```python
from build123d import *

# Parameters (mm, degrees)
SKETCH16_R             = 3.4
SKETCH16_R_2           = 3
MEMBER_1_DEPTH         = 340
HOLE_WIZARD_M8_3_D     = 6.9
HOLE_WIZARD_M8_3_DEPTH = 19.75
HOLE_WIZARD_M8_3_TIP   = 2.072969136


with BuildPart() as part:
    # Sketch16 → Member 1 (new body)
    with BuildSketch(Plane(origin=(0, 0, 0), x_dir=(-1, 0, 0), z_dir=(0, 1, 0))):
        with BuildLine():
            Line((-5.1, 20), (-5.1, 19.5))
            Line((-5.1, 19.5), (-4.1, 19.5))
            Line((-4.1, 19.5), (-4.1, 17))
            Line((-4.1, 17), (-6.1, 17))
            Line((-6.1, 17), (-6.1, 18))
            Line((-6.1, 18), (-10.3, 18))
            Line((-10.3, 18), (-10.3, 12))
            Line((-10.3, 12), (-6, 7.7))
            Line((-6, 7.7), (6, 7.7))
            Line((6, 7.7), (10.3, 12))
            Line((10.3, 12), (10.3, 18))
            Line((10.3, 18), (6.1, 18))
            Line((6.1, 18), (6.1, 17))
            Line((6.1, 17), (4.1, 17))
            Line((4.1, 17), (4.1, 19.5))
            Line((4.1, 19.5), (5.1, 19.5))
            Line((5.1, 19.5), (5.1, 20))
            Line((5.1, 20), (15.5, 20))
            ThreePointArc((15.5, 20), (18.681980515, 18.681980515), (20, 15.5))
            Line((20, 15.5), (20, 5.1))
            Line((20, 5.1), (19.5, 5.1))
            Line((19.5, 5.1), (19.5, 4.1))
            Line((19.5, 4.1), (17, 4.1))
            Line((17, 4.1), (17, 6.1))
            Line((17, 6.1), (18, 6.1))
            Line((18, 6.1), (18, 10.3))
            Line((18, 10.3), (12, 10.3))
            Line((12, 10.3), (7.7, 6))
            Line((7.7, 6), (7.7, -6))
            Line((7.7, -6), (12, -10.3))
            Line((12, -10.3), (18, -10.3))
            Line((18, -10.3), (18, -6.1))
            Line((18, -6.1), (17, -6.1))
            Line((17, -6.1), (17, -4.1))
            Line((17, -4.1), (19.5, -4.1))
            Line((19.5, -4.1), (19.5, -5.1))
            Line((19.5, -5.1), (20, -5.1))
            Line((20, -5.1), (20, -15.5))
            ThreePointArc((20, -15.5), (18.681980515, -18.681980515), (15.5, -20))
            Line((15.5, -20), (5.1, -20))
            Line((5.1, -20), (5.1, -19.5))
            Line((5.1, -19.5), (4.1, -19.5))
            Line((4.1, -19.5), (4.1, -17))
            Line((4.1, -17), (6.1, -17))
            Line((6.1, -17), (6.1, -18))
            Line((6.1, -18), (10.3, -18))
            Line((10.3, -18), (10.3, -12))
            Line((10.3, -12), (6, -7.7))
            Line((6, -7.7), (-6, -7.7))
            Line((-6, -7.7), (-10.3, -12))
            Line((-10.3, -12), (-10.3, -18))
            Line((-10.3, -18), (-6.1, -18))
            Line((-6.1, -18), (-6.1, -17))
            Line((-6.1, -17), (-4.1, -17))
            Line((-4.1, -17), (-4.1, -19.5))
            Line((-4.1, -19.5), (-5.1, -19.5))
            Line((-5.1, -19.5), (-5.1, -20))
            Line((-5.1, -20), (-15.5, -20))
            ThreePointArc((-15.5, -20), (-18.681980515, -18.681980515), (-20, -15.5))
            Line((-20, -15.5), (-20, -5.1))
            Line((-20, -5.1), (-19.5, -5.1))
            Line((-19.5, -5.1), (-19.5, -4.1))
            Line((-19.5, -4.1), (-17, -4.1))
            Line((-17, -4.1), (-17, -6.1))
            Line((-17, -6.1), (-18, -6.1))
            Line((-18, -6.1), (-18, -10.3))
            Line((-18, -10.3), (-12, -10.3))
            Line((-12, -10.3), (-7.7, -6))
            Line((-7.7, -6), (-7.7, 6))
            Line((-7.7, 6), (-12, 10.3))
            Line((-12, 10.3), (-18, 10.3))
            Line((-18, 10.3), (-18, 6.1))
            Line((-18, 6.1), (-17, 6.1))
            Line((-17, 6.1), (-17, 4.1))
            Line((-17, 4.1), (-19.5, 4.1))
            Line((-19.5, 4.1), (-19.5, 5.1))
            Line((-19.5, 5.1), (-20, 5.1))
            Line((-20, 5.1), (-20, 15.5))
            ThreePointArc((-20, 15.5), (-18.681980515, 18.681980515), (-15.5, 20))
            Line((-15.5, 20), (-5.1, 20))
        make_face()
        Circle(SKETCH16_R, mode=Mode.SUBTRACT)
        with Locations((-15.556349186, 15.556349186)):
            Circle(SKETCH16_R_2, mode=Mode.SUBTRACT)
        with Locations((15.556349186, 15.556349186)):
            Circle(SKETCH16_R_2, mode=Mode.SUBTRACT)
        with Locations((15.556349186, -15.556349186)):
            Circle(SKETCH16_R_2, mode=Mode.SUBTRACT)
        with Locations((-15.556349186, -15.556349186)):
            Circle(SKETCH16_R_2, mode=Mode.SUBTRACT)
    extrude(amount=MEMBER_1_DEPTH)

    # M8 螺纹孔3
    with Locations(Plane(origin=(0, 340, 0), x_dir=(1, 0, 0), z_dir=(0, 1, 0))):
        with Locations((0, 0)):
            Hole(HOLE_WIZARD_M8_3_D / 2, depth=HOLE_WIZARD_M8_3_DEPTH)
            with Locations((0, 0, -(HOLE_WIZARD_M8_3_DEPTH + HOLE_WIZARD_M8_3_TIP / 2))):  # 118° drill point
                Cone(0, HOLE_WIZARD_M8_3_D / 2, HOLE_WIZARD_M8_3_TIP, mode=Mode.SUBTRACT)


solid = part.part
```
Input: part model. Units: mm. Frame: model coordinates. A direction names the side the tool comes from. Give positions to 0.01 mm unless a question says otherwise; leave off trailing zeros. Order: outer loops, then holes, each group sorted by start corner. A loop starts at its lowest first (then second) coordinate and runs counter-clockwise, first axis right, second up. Notation, with made-up numbers: (79.5, 10.5) - (137.5, 10.5) arc R11 cw to (137.5, 26.5) - close; hole circle Ø7 at (70.5, 38.5). An arc over 180 degrees is marked (long way). Use a Markdown table: item, result.
(1) Section query A-A (z = 0). Output: boundary loops of the cut face in (x, y), then the cut area to 3 significant figures.
Computed values:
| item | result |
|---|---|
| outline | (-7.7, 0) - (-3.4, 0) - (-3.4, 320.22) - (-3.45, 320.25) - (-3.45, 340) - (-7.7, 340) - close; (3.4, 0) - (7.7, 0) - (7.7, 340) - (3.45, 340) - (3.45, 320.25) - (3.4, 320.22) - close |
| area | 2,920 mm2 |
(2) Section query C-C (y = 153). State how many separate pieces and enclosed holes the cut face has, then the cut area to 3 significant figures.
Computed values:
| item | result |
|---|---|
| separate pieces | 1 |
| enclosed holes | 5 |
| area | 605 mm2 |
(3) Access query for faces 4 (the flat face through (15, 168, 10.3)), 5 (the flat face through (10, 168, 20)). Directions: +Z, -Z, +X, -X, +Y, -Y. A direction counts if a zero-diameter tool reaches every point of the face in a straight line with its end or side. Return the directions, or none.
Computed values:
| item | result |
|---|---|
| face 4 | +Y, -Y |
| face 5 | +Z, +X, -X, +Y, -Y |
(4) Pin query (flat end, axial travel): pin 1 (2 mm diameter, centred on y = 172.5, z = -18, fed in from -X); pin 2 (1.1 mm diameter, centred on x = 17.5, y = 143, fed in from -Z); pin 3 (1.5 mm diameter, centred on x = -3, y = 154, fed in from -Z); pin 4 (6 mm diameter, centred on x = -9.5, z = -3, fed in from +Y). Return the tip coordinate at first contact, or that it passes through.
Computed values:
| item | result |
|---|---|
| pin 1 | stops at x = -19.74 |
| pin 2 | stops at z = -19.76 |
| pin 3 | stops at z = -7.7 |
| pin 4 | stops at y = 340 |
(5) Section query B-B (x = 0). Output: boundary loops of the cut face in (y, z), then the cut area to 3 significant figures.
Computed values:
| item | result |
|---|---|
| outline | (0, -7.7) - (340, -7.7) - (340, -3.45) - (320.25, -3.45) - (320.22, -3.4) - (0, -3.4) - close; (0, 3.4) - (320.22, 3.4) - (320.25, 3.45) - (340, 3.45) - (340, 7.7) - (0, 7.7) - close |
| area | 2,920 mm2 |
(6) Line query: line 1 (Z direction, x = 12.5, y = 318); line 2 (X direction, y = 298, z = 8.5); line 3 (Z direction, x = 0, y = 62). Output: solid intervals per line, ascending. Write a range as from..to.
Computed values:
| item | result |
|---|---|
| line 1 | z = -20..-10.3, 10.3..20 |
| line 2 | x = -20..-18, -10.2..-6.8, 6.8..10.2, 18..20 |
| line 3 | z = -7.7..-3.4, 3.4..7.7 |
(7) Draft query along Z for faces 1 (the flat face through (10, 168, -20)), 2 (the cylindrical face through (15.95, 167.62, 18.53)), 3 (the flat face through (-10, 168, 20)). Return one class per face: released by +Z, released by -Z, zero draft, split by the parting line, or undercut.
Computed values:
| item | result |
|---|---|
| face 1 | released by -Z |
| face 2 | undercut |
| face 3 | released by +Z |
